Part model, mm, in its own coordinate system. A direction names the side the tool comes from. Round coordinates to 2 decimals unless told otherwise and drop trailing zeros. Loops run counter-clockwise (first coordinate to the right, second up) from the corner with the lowest first, then second, coordinate; pieces in that order, holes last. Notation, with made-up numbers: M 75.25,56.25 L 115.25,56.25 A18 cw 115.25,75.25 Z; hole C -5.5,88.5 d9. An arc over 180 degrees is marked long. Write each question's results on one line, items separated by ' | '.
from build123d import *

# Parameters (mm, degrees)
SKETCH1_W                                        = 120
SKETCH1_H                                        = 65
BOSS_EXTRUDE1_DEPTH                              = 12
HOLE_FOR_TORX_SOCKET_CAP_SCREW1_D                = 11
HOLE_FOR_TORX_SOCKET_CAP_SCREW1_CBORE_D          = 18
HOLE_FOR_TORX_SOCKET_CAP_SCREW1_CBORE_DEPTH      = 7
HOLE_FOR_SOCKET_HEAD_CAP_SCREW_TYPE2_D           = 5.5
HOLE_FOR_SOCKET_HEAD_CAP_SCREW_TYPE2_CBORE_D     = 10
HOLE_FOR_SOCKET_HEAD_CAP_SCREW_TYPE2_CBORE_DEPTH = 5.7


with BuildPart() as part:
    # Sketch1 → Boss-Extrude1 (new body)
    with BuildSketch(Plane.XY):
        Rectangle(SKETCH1_W, SKETCH1_H)
    extrude(amount=BOSS_EXTRUDE1_DEPTH)

    # Hole for Torx socket cap screw1 (through all)
    with Locations(Plane.XY.offset(12)):
        with Locations((-38, 0), (38, 0)):
            CounterBoreHole(HOLE_FOR_TORX_SOCKET_CAP_SCREW1_D / 2, HOLE_FOR_TORX_SOCKET_CAP_SCREW1_CBORE_D / 2, HOLE_FOR_TORX_SOCKET_CAP_SCREW1_CBORE_DEPTH)

    # Hole for socket head cap screw, type2 (through all)
    with Locations(Plane(origin=(0, 0, 0), x_dir=(-1, 0, 0), z_dir=(0, 0, -1))):
        with Locations((-37, 15), (-37, -15), (37, -15), (37, 15)):
            CounterBoreHole(HOLE_FOR_SOCKET_HEAD_CAP_SCREW_TYPE2_D / 2, HOLE_FOR_SOCKET_HEAD_CAP_SCREW_TYPE2_CBORE_D / 2, HOLE_FOR_SOCKET_HEAD_CAP_SCREW_TYPE2_CBORE_DEPTH)


solid = part.part
Item 1: Two-plate mould, pull along X, no slides. Class faces 4 (the flat face through (-60, 0, 6)), 5 (the cylindrical face through (-32.505, 0.242, 2.465)), 6 (the flat face through (-1, 0, 0)): +X half, -X half, draft (parallel to the pull), parting line (faces both ways), or undercut.
Filled sheet:
face 4: -X half | face 5: undercut | face 6: draft
Item 2: Band-saw the part on C-C on x = -37. Give the cut face in (y, z), and give its area (3 significant figures).
Filled sheet:
outline: M -32.5,0 L -20,0 L -20,5.7 L -17.75,5.7 L -17.75,12 L -32.5,12 Z; M -12.25,5.7 L -10,5.7 L -10,0 L -5.41,0 L -5.41,5 L -8.94,5 L -8.94,12 L -12.25,12 Z; M 5.41,0 L 10,0 L 10,5.7 L 12.25,5.7 L 12.25,12 L 8.94,12 L 8.94,5 L 5.41,5 Z; M 17.75,5.7 L 20,5.7 L 20,0 L 32.5,0 L 32.5,12 L 17.75,12 Z | area: 417 mm^2
Item 3: Which spindle directions (+Z, -Z, +X, -X, +Y, -Y) get a long thin tool onto all of the face, cutting with end or side? Do faces 1 (the cylindrical face through (-33, 12, 3)), 2 (the flat face through (42, 4, 5)), 3 (the flat face through (-1, 32.5, 6)). Say none if no direction does.
Filled sheet:
face 1: -Z | face 2: +Z | face 3: +Z, -Z, +X, -X, +Y
Item 4: Wall check: L1, parallel to X at y = -1, z = 9.75; L2, parallel to Y at x = 37, z = 3.6; L3, parallel to X at y = -14.5, z = 6. Give the ranges that are in metal, low to high.
Filled sheet:
L1: -60 to -46.94, -29.06 to 29.06, 46.94 to 60 | L2: -32.5 to -20, -10 to -5.41, 5.41 to 10, 20 to 32.5 | L3: -60 to -39.7, -34.3 to 34.3, 39.7 to 60
Item 5: Band-saw the part on A-A on z = 9.25. Give the cut face in (x, y).
Filled sheet:
outline: M -60,-32.5 L 60,-32.5 L 60,32.5 L -60,32.5 Z; hole C -38,0 d18; hole C -37,-15 d5.5; hole C -37,15 d5.5; hole C 38,0 d18; hole C 37,-15 d5.5; hole C 37,15 d5.5
Item 6: Band-saw the part on B-B on y = 15. Give the cut face in (x, z), and give its area (3 significant figures).
Filled sheet:
outline: M -60,0 L -42,0 L -42,5.7 L -39.75,5.7 L -39.75,12 L -60,12 Z; M -34.25,5.7 L -32,5.7 L -32,0 L 32,0 L 32,5.7 L 34.25,5.7 L 34.25,12 L -34.25,12 Z; M 39.75,5.7 L 42,5.7 L 42,0 L 60,0 L 60,12 L 39.75,12 Z | area: 1,260 mm^2
Item 7: Drop a flat-ended pin along its axis: P1, Ø5, axis at x = 36.5, y = -16.5, coming from the -Z side. Give the stop position or say it passes through.
Filled sheet:
P1: z = 5.7
